Design review of the part built by this model. Coordinates are the model's own, in mm. A direction names the side the tool comes from. Coordinates: 2 decimals unless noted, no trailing zeros. Write each loop counter-clockwise with the first axis right and the second up, starting at its lowest first coordinate (ties: lowest second). Pieces come first, ordered by that corner, then holes. Notation, with made-up numbers: (-2, 89.25) - (34, 89.25) arc R8 ccw to (34, 93.25) - close; hole circle Ø9 at (8, -28.75). An arc over 180 degrees is marked (long way). Answer as CSV lines item,"result". Start each with the question number.
Q1. For line 1 along X through (y, z) = (3, -1.75); line 2 along Z through (x, y) = (-9, -1); line 3 along Z through (x, y) = (-7, 1), list the stretches that pass through material, from the lowest coordinate up. Write a range as [from, to].
Q2. Machinability: for faces 1 (the face through (-15, -1, 0)), 2 (the face through (-0.168, -11.86, -3.386)), 3 (the face through (0.168, -11.86, 3.386)), which of the approach directions +Z, -Z, +X, -X, +Y, -Y give a long, thin tool a straight path to every point of the face, cutting with its end or side? Answer none if there is none.
Q3. We need section B-B (z = 0). Write out the cut boundary in (x, y).
Q4. We need section C-C (z = 2.5). State how many separate pieces and enclosed holes the cut face has, plus the area to 3 significant figures.
Q5. We need section A-A (y = 4). Write out the cut boundary in (x, z).
Q6. Clearance check with flat-ended pins moving along their axes: pin 1 (6 mm diameter, centred on x = -10, y = -9.5, fed in from +Z); pin 2 (4 mm diameter, centred on y = 1.5, z = -3.5, fed in from +X); pin 3 (2 mm diameter, centred on x = -0.5, y = -0.5, fed in from -Z); pin 4 (6 mm diameter, centred on x = -8.5, y = -6.5, fed in from -Z). State where each tip first meets the part, or that it passes through.
Q7. Mouldability with a two-part tool opening along X and no side actions: class faces 4 (the face through (-13.476, 3.368, 0.049)), 5 (the face through (0, 10, 0)), 6 (the face through (25, 5, 0)) as pulls with the +X half, pulls with the -X half, needs draft (parallel to the pull), parting line crosses it, or undercut.
from build123d import *

# Parameters (mm, degrees)
SKETCH_1_3_W          = 50
SKETCH_1_3_H          = 7
BOSS_EXTRUDE1_DEPTH   = 10
BOSS_EXTRUDE2_DEPTH   = 2
BOSS_EXTRUDE3_DEPTH   = 20
BOSS_EXTRUDE3_DRAFT   = -8
FILLET1_R             = 2
M4_TAPPED_HOLE1_D     = 3.3
M4_TAPPED_HOLE1_DEPTH = 10.1
M4_TAPPED_HOLE1_TIP   = 0.991420021


with BuildPart() as part:
    # Sketch 1_3 → Boss-Extrude1 (new body)
    with BuildSketch(Plane(origin=(0, 0, 0), x_dir=(1, 0, 0), z_dir=(0, 1, 0))):
        Rectangle(SKETCH_1_3_W, SKETCH_1_3_H)
    extrude(amount=BOSS_EXTRUDE1_DEPTH)

    # Sketch 1_3 2 → Boss-Extrude2 (add)
    with BuildSketch(Plane(origin=(0, 0, 0), x_dir=(1, 0, 0), z_dir=(0, 1, 0))):
        with BuildLine():
            Line((-12, 3), (12, 3))
            ThreePointArc((12, 3), (15, 0), (12, -3))
            Line((12, -3), (-12, -3))
            ThreePointArc((-12, -3), (-15, 0), (-12, 3))
        make_face()
    extrude(amount=-BOSS_EXTRUDE2_DEPTH)


with BuildPart() as boss_extrude3_tool:
    # Sketch2 → Boss-Extrude3 (with draft: the straight prism first)
    with BuildSketch(Plane.XZ.offset(2)):
        with BuildLine():
            Line((12, 2), (-12, 2))
            ThreePointArc((-12, 2), (-14, 0), (-12, -2))
            Line((-12, -2), (12, -2))
            ThreePointArc((12, -2), (14, 0), (12, 2))
        make_face()
    extrude(amount=BOSS_EXTRUDE3_DEPTH)
    # Boss-Extrude3: the draft: its side faces are tilted about the plane it starts from
    boss_extrude3_sides = [boss_extrude3_tool.faces().sort_by_distance(p)[0] for p in [
        (0, -12, 2),
        (-14, -12, 0),
        (0, -12, -2),
        (14, -12, 0),
    ]]
    draft(boss_extrude3_sides, Plane.XZ.offset(2), BOSS_EXTRUDE3_DRAFT)


with BuildPart() as part_1:
    add(part.part)

    # Boss-Extrude3: add boss_extrude3_tool
    add(boss_extrude3_tool.part)

    # Fillet1
    fillet1_edges = [part_1.edges().sort_by_distance(p)[0] for p in [
        (-25, 5, 3.5),
        (-25, 5, -3.5),
        (25, 5, -3.5),
        (25, 5, 3.5),
    ]]
    fillet(fillet1_edges, radius=FILLET1_R)

    # M4 Tapped Hole1
    with Locations(Plane(origin=(15, 4, -3.5), x_dir=(-1, 0, 0), z_dir=(0, 0, -1))):
        with Locations((0, 0), (30, 0)):
            Hole(M4_TAPPED_HOLE1_D / 2, depth=M4_TAPPED_HOLE1_DEPTH)
            with Locations((0, 0, -(M4_TAPPED_HOLE1_DEPTH + M4_TAPPED_HOLE1_TIP / 2))):  # 118° drill point
                Cone(0, M4_TAPPED_HOLE1_D / 2, M4_TAPPED_HOLE1_TIP, mode=Mode.SUBTRACT)


solid = part_1.part
Results list:
1,line 1,"x = [-24.98, -16.31], [-13.69, 13.69], [16.31, 24.98]"
1,line 2,"z = [-3, 3]"
1,line 3,"z = [-3.5, 3.5]"
2,face 1,"-X"
2,face 2,"-Z, +X, -X"
2,face 3,"+Z, +X, -X"
3,outline,"(-25, 0) - (-15, 0) - (-15, -2) - (-14, -2) - (-16.81, -22) - (16.81, -22) - (14, -2) - (15, -2) - (15, 0) - (25, 0) - (25, 10) - (-25, 10) - close; hole circle Ø3.3 at (-15, 4); hole circle Ø3.3 at (15, 4)"
4,separate pieces,"2"
4,enclosed holes,"2"
4,area,"1,010 mm2"
5,outline,"(-25, -1.5) arc R2 ccw to (-23, -3.5) - (-16.65, -3.5) - (-16.65, 3.5) - (-23, 3.5) arc R2 ccw to (-25, 1.5) - close; (-13.35, -3.5) - (13.35, -3.5) - (13.35, 3.5) - (-13.35, 3.5) - close; (16.65, -3.5) - (23, -3.5) arc R2 ccw to (25, -1.5) - (25, 1.5) arc R2 ccw to (23, 3.5) - (16.65, 3.5) - close"
6,pin 1,"stops at z = 3.48"
6,pin 2,"stops at x = 25"
6,pin 3,"stops at z = -3.5"
6,pin 4,"stops at z = -3.05"
7,face 4,"undercut"
7,face 5,"needs draft"
7,face 6,"pulls with the +X half"
